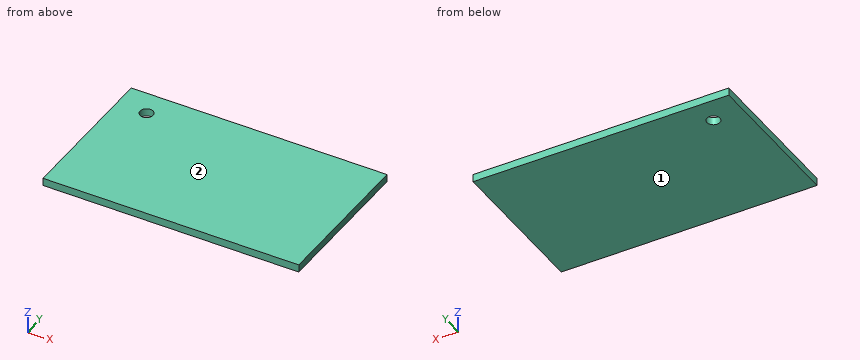
```python
from build123d import *

# Parameters (mm, degrees)
SKETCH1_W              = 200
SKETCH1_H              = 120
BOSS_EXTRUDE1_DEPTH    = 6
M12_TAPPED_HOLE1_D     = 10.2
M12_TAPPED_HOLE1_DEPTH = 29.25
M12_TAPPED_HOLE1_TIP   = 3.064389157


with BuildPart() as part:
    # Sketch1 → Boss-Extrude1 (new body)
    with BuildSketch(Plane.XY):
        Rectangle(SKETCH1_W, SKETCH1_H)
    extrude(amount=BOSS_EXTRUDE1_DEPTH)

    # M12 Tapped Hole1
    with Locations(Plane.XY.offset(6)):
        with Locations((-76.5, 40)):
            Hole(M12_TAPPED_HOLE1_D / 2, depth=M12_TAPPED_HOLE1_DEPTH)
            with Locations((0, 0, -(M12_TAPPED_HOLE1_DEPTH + M12_TAPPED_HOLE1_TIP / 2))):  # 118° drill point
                Cone(0, M12_TAPPED_HOLE1_D / 2, M12_TAPPED_HOLE1_TIP, mode=Mode.SUBTRACT)


solid = part.part
```
CAD build for the part. Positions are in the model's coordinates, mm. Face numbers are marked on the shaded views. Round coordinates to 2 decimals unless told otherwise and drop trailing zeros. Order: outer loops, then holes, each group sorted by start corner. A loop starts at its lowest first (then second) coordinate and runs counter-clockwise, first axis right, second up. Notation, with made-up numbers: (47, -28.5) - (73, -28.5) arc R28 ccw to (73, 5.5) - close; hole circle Ø4 at (13.25, 34). An arc over 180 degrees is marked (long way). Answer in a Markdown table with one row per item. Add a question column.
(1) Mould opens along Z. For the marked faces 1 and 2 say: +Z half, -Z half, draft (parallel to the pull), parting line (faces both ways), or undercut.
(2) Band-saw the part on B-B on x = -76.5. List the corners of the cut face in (y, z), and give its area (3 significant figures).
(3) Band-saw the part on A-A on y = 40. List the corners of the cut face in (x, z), and give its area (3 significant figures).
(4) Probe L1, parallel to Y at x = -76.5, z = 1.8; L2, parallel to X at y = 37.5, z = 2.15. List the from-to ranges inside material, lowest first. Write a range as [from, to].
Data:
| question | item | result |
|---|---|---|
| 1 | face 1 | -Z half |
| 1 | face 2 | +Z half |
| 2 | outline | (-60, 0) - (34.9, 0) - (34.9, 6) - (-60, 6) - close; (45.1, 0) - (60, 0) - (60, 6) - (45.1, 6) - close |
| 2 | area | 659 mm^2 |
| 3 | outline | (-100, 0) - (-81.6, 0) - (-81.6, 6) - (-100, 6) - close; (-71.4, 0) - (100, 0) - (100, 6) - (-71.4, 6) - close |
| 3 | area | 1,140 mm^2 |
| 4 | L1 | y = [-60, 34.9], [45.1, 60] |
| 4 | L2 | x = [-100, -80.95], [-72.05, 100] |
